Input: dimensioned drawing with shaded views. Units: mm. Origin: part minimum x, y, z. A direction names the side the tool comes from. Give positions to 0.01 mm unless a question says otherwise; leave off trailing zeros. Order: outer loops, then holes, each group sorted by start corner. A loop starts at its lowest first (then second) coordinate and runs counter-clockwise, first axis right, second up. Notation, with made-up numbers: M -38.5,-4 L -27.5,-4 A17 ccw -27.5,19 Z; hole C 81.5,2 d7. An arc over 180 degrees is marked long. Answer in a Markdown table with one row per item. Add a question column.
(1) Section query A-A, the plane x = 12. Return loops of the section in (y, z), plus the area to 3 significant figures.
(2) Section query C-C, the plane y = 26. Return loops of the section in (x, z), plus the area to 3 significant figures.
(3) Section query B-B, the plane z = 125. Return loops of the section in (x, y).
(4) Mould query, pull axis X, two halves, no side actions, for the marked faces 1, 2, 3 and 4. Classes: pulls with the +X half, pulls with the -X half, needs draft (parallel to the pull), parting line crosses it, or undercut.
(5) Pin query (flat end, axial travel): P1, Ø10, axis at x = 5.5, y = 37, coming from the -Z side. Return the tip coordinate at first contact, or that it passes through.
(6) Material intervals for line 1 along X through (y, z) = (15.5, 131); line 2 along Y through (x, z) = (26, 18), sorted ascending.
(7) Set-up query: the marked faces 5 and 6. Return all of +Z, -Z, +X, -X, +Y, -Y with unobstructed straight access to the full face (end or side cutting, diameter ignored); none if empty.
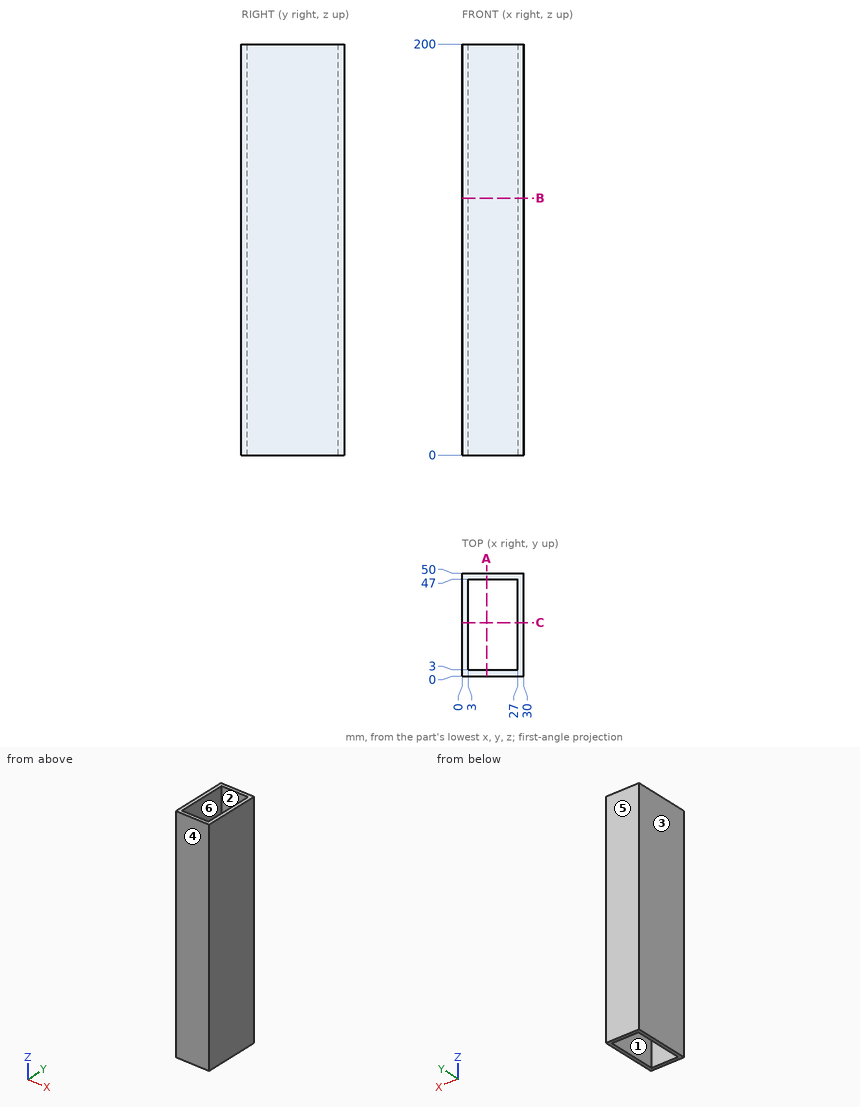
Values follow:
| question | item | result |
|---|---|---|
| 1 | outline | M 0,0 L 3,0 L 3,200 L 0,200 Z; M 47,0 L 50,0 L 50,200 L 47,200 Z |
| 1 | area | 1,200 mm² |
| 2 | outline | M 0,0 L 3,0 L 3,200 L 0,200 Z; M 27,0 L 30,0 L 30,200 L 27,200 Z |
| 2 | area | 1,200 mm² |
| 3 | outline | M 0,0 L 30,0 L 30,50 L 0,50 Z; hole M 3,3 L 27,3 L 27,47 L 3,47 Z |
| 4 | face 1 | undercut |
| 4 | face 2 | undercut |
| 4 | face 3 | pulls with the -X half |
| 4 | face 4 | needs draft |
| 5 | P1 | stops at z = 0 |
| 6 | line 1 | x = 0 to 3, 27 to 30 |
| 6 | line 2 | y = 0 to 3, 47 to 50 |
| 7 | face 5 | +Z, -Z, +X, -X, +Y |
| 7 | face 6 | +Z, -Z |
